The listing builds one solid part. Answer for the finished solid, in the listing's coordinates (mm). Coordinates: 2 decimals unless noted, no trailing zeros. Write each loop counter-clockwise with the first axis right and the second up, starting at its lowest first coordinate (ties: lowest second). Pieces come first, ordered by that corner, then holes.
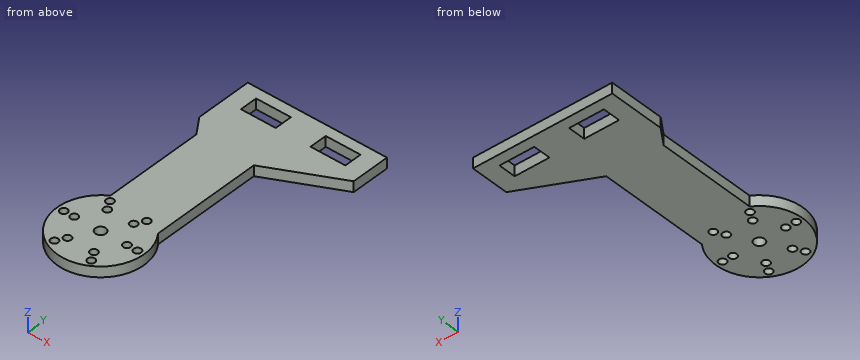
from build123d import *

# Parameters (mm, degrees)
SKETCH_1_R      = 1.5
SKETCH_1_R_2    = 1.075
SKETCH_1_W      = 10
SKETCH_1_H      = 5
EXTRUDE_1_DEPTH = 3


with BuildPart() as part:
    # 草图1 → 凸台-拉伸1 (new body)
    with BuildSketch(Plane.XY):
        with BuildLine():
            Line((-15.405029449, -13.33425996), (-15.405029449, 15.090143764))
            Line((-15.405029449, 15.090143764), (-18.905029449, 20.088661788))
            Line((-18.905029449, 20.088661788), (-18.905029449, 36.088661788))
            Line((-18.905029449, 36.088661788), (21.094970551, 36.088661788))
            Line((21.094970551, 36.088661788), (21.094970551, 25.088661788))
            Line((21.094970551, 25.088661788), (1.094970551, 15.088661788))
            Line((1.094970551, 15.088661788), (1.094970551, -16.511338212))
            ThreePointArc((1.094970551, -16.511338212), (-11.26849228, -36.285866449), (-15.405029449, -13.33425996))
        make_face()
        with Locations((-8.905029449, -24.011338212)):
            Circle(SKETCH_1_R, mode=Mode.SUBTRACT)
        with Locations((-1.325029449, -24.011338212)):
            Circle(SKETCH_1_R_2, mode=Mode.SUBTRACT)
        with Locations((1.674970551, -24.011338212)):
            Circle(SKETCH_1_R_2, mode=Mode.SUBTRACT)
        with Locations((-5.115029449, -30.575810773)):
            Circle(SKETCH_1_R_2, mode=Mode.SUBTRACT)
        with Locations((-3.615029449, -33.173886984)):
            Circle(SKETCH_1_R_2, mode=Mode.SUBTRACT)
        with Locations((-12.695029449, -30.575810773)):
            Circle(SKETCH_1_R_2, mode=Mode.SUBTRACT)
        with Locations((-14.195029449, -33.173886984)):
            Circle(SKETCH_1_R_2, mode=Mode.SUBTRACT)
        with Locations((-16.485029449, -24.011338212)):
            Circle(SKETCH_1_R_2, mode=Mode.SUBTRACT)
        with Locations((-19.485029449, -24.011338212)):
            Circle(SKETCH_1_R_2, mode=Mode.SUBTRACT)
        with Locations((-12.695029449, -17.446865652)):
            Circle(SKETCH_1_R_2, mode=Mode.SUBTRACT)
        with Locations((-14.195029449, -14.84878944)):
            Circle(SKETCH_1_R_2, mode=Mode.SUBTRACT)
        with Locations((-5.115029449, -17.446865652)):
            Circle(SKETCH_1_R_2, mode=Mode.SUBTRACT)
        with Locations((-3.615029449, -14.84878944)):
            Circle(SKETCH_1_R_2, mode=Mode.SUBTRACT)
        with Locations((-8.905029449, 30.588661788)):
            Rectangle(SKETCH_1_W, SKETCH_1_H, mode=Mode.SUBTRACT)
        with Locations((11.094970551, 30.588661788)):
            Rectangle(SKETCH_1_W, SKETCH_1_H, mode=Mode.SUBTRACT)
    extrude(amount=EXTRUDE_1_DEPTH)


solid = part.part
1. Section D-D on x = -1.5 is taken. Give the vertices of the cut face in (y, z), then the cut area to 3 significant figures.
Results found:
outline: (-34.08, 0) - (-25.07, 0) - (-25.07, 3) - (-34.08, 3) - close; (-22.95, 0) - (36.09, 0) - (36.09, 3) - (-22.95, 3) - close
area: 204 mm2
2. Section A-A on y = 29.5 is taken. Give the vertices of the cut face in (x, z), then the cut area to 3 significant figures.
Results found:
outline: (-18.91, 0) - (-13.91, 0) - (-13.91, 3) - (-18.91, 3) - close; (-3.91, 0) - (6.09, 0) - (6.09, 3) - (-3.91, 3) - close; (16.09, 0) - (21.09, 0) - (21.09, 3) - (16.09, 3) - close
area: 60.0 mm2
3. Section C-C on z = 1.55 is taken. State how many separate pieces and enclosed holes the cut face has, then the cut area to 3 significant figures.
Results found:
separate pieces: 1
enclosed holes: 15
area: 1,530 mm2
4. Find the intervals of material crossed by L1, parallel to X at y = -24.5, z = 0.5; L2, parallel to X at y = -30, z = 2.7; L3, parallel to X at y = -13, z = 1.2, in increasing order.
Results found:
L1: x = -21.4 to -20.44, -18.53 to -17.44, -15.53 to -10.32, -7.49 to -2.28, -0.37 to 0.72, 2.63 to 3.59
L2: x = -19.88 to -13.6, -11.79 to -6.02, -4.21 to 2.07
L3: x = -15.41 to 1.09
5. Section B-B on x = 14 is taken. Give the vertices of the cut face in (y, z), then the cut area to 3 significant figures.
Results found:
outline: (21.54, 0) - (28.09, 0) - (28.09, 3) - (21.54, 3) - close; (33.09, 0) - (36.09, 0) - (36.09, 3) - (33.09, 3) - close
area: 28.6 mm2
6. Flat-ended cylindrical pins translate along their axes: P1, Ø3.5, axis at x = -14.2, y = -14.85, coming from the -Z side; P2, Ø1.5, axis at y = 31.5, z = 1.5, coming from the -X side (3 decimals); P3, Ø1.5, axis at x = 12.5, z = 1.5, coming from the -Y side; P4, Ø1.5, axis at y = -26.5, z = 1.5, coming from the +X side. Find the tip coordinate at first contact, or state that the pin passes through.
Results found:
P1: stops at z = 0
P2: stops at x = -18.905
P3: stops at y = 20.42
P4: stops at x = 3.47
